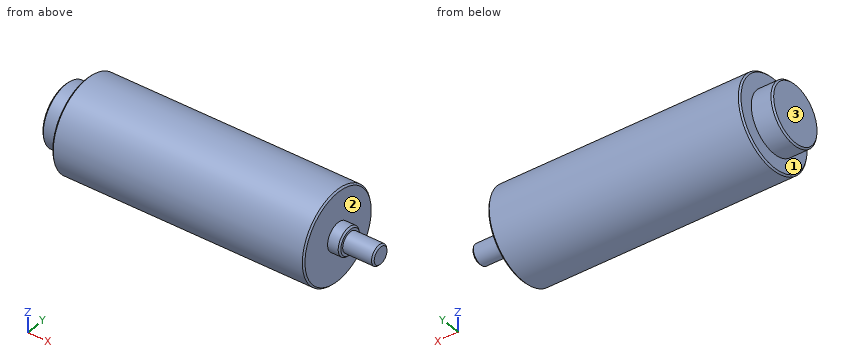
from build123d import *

# Parameters (mm, degrees)
CHAMFER1_SIZE = 0.5


with BuildPart() as part:
    # Sketch1 → Revolve1 (revolve)
    with BuildSketch(Plane.XY):
        Polygon((695.508784709, 30.649610335), (685.508784709, 30.649610335), (685.508784709, 31.949610335), (681.508784709, 31.949610335), (681.508784709, 42.349610335), (598.508784709, 42.349610335), (598.508784709, 37.349610335), (591.508784709, 37.349610335), (591.508784709, 27.349610335), (695.508784709, 27.349610335), align=None)
    revolve(axis=Axis((695.508784709, 27.349610335, 0), (-1, 0, 0)))

    # Chamfer1
    chamfer1_edges = [part.edges().sort_by_distance(p)[0] for p in [
        (695.508784709, 24.049610335, 0),
        (685.508784709, 22.749610335, 0),
        (681.508784709, 12.349610335, 0),
        (598.508784709, 12.349610335, 0),
        (591.508784709, 17.349610335, 0),
    ]]
    chamfer(chamfer1_edges, length=CHAMFER1_SIZE)


solid = part.part
Geometry check sheet. Reference: the model listing, model coordinates, mm. Face numbers are marked on the shaded views. A direction names the side the tool comes from. Give positions to 0.01 mm unless a question says otherwise; leave off trailing zeros. Loops run counter-clockwise (first coordinate to the right, second up) from the corner with the lowest first, then second, coordinate; pieces in that order, holes last.
(1) Thickness scan on L1, parallel to X at y = 25, z = 3; L2, parallel to Y at x = 661.5, z = -0.5; L3, parallel to X at y = 21.5, z = -12.5. Record the ranges inside material, lowest first.
From the geometry:
L1: x = 591.51 to 685.51
L2: y = 12.36 to 42.34
L3: x = 598.51 to 681.51
(2) Set-up check for the marked faces 1, 2 and 3: record each of +Z, -Z, +X, -X, +Y, -Y from which the full face is reachable in a straight line by a thin tool's end or side.
From the geometry:
face 1: -X
face 2: +X
face 3: +Z, -Z, -X, +Y, -Y
(3) Depth check by flat-ended pin: pin 1 Ø2 at (x, y) = (655, 29.5) entering from -Z; pin 2 Ø1 at (x, y) = (672.5, 36.5) entering from -Z; pin 3 Ø1.5 at (x, z) = (652, 11.5) entering from -Y. Enter the tip coordinate at first touch or a pass-through.
From the geometry:
pin 1: stops at z = -14.96
pin 2: stops at z = -12.25
pin 3: stops at y = 16.89
(4) Section check A-A on z = 0. Record the cut outline in (x, y), then the cut area to 3 significant figures.
From the geometry:
outline: (591.51, 17.85) - (592.01, 17.35) - (598.51, 17.35) - (598.51, 12.85) - (599.01, 12.35) - (681.01, 12.35) - (681.51, 12.85) - (681.51, 22.75) - (685.01, 22.75) - (685.51, 23.25) - (685.51, 24.05) - (695.01, 24.05) - (695.51, 24.55) - (695.51, 30.15) - (695.01, 30.65) - (685.51, 30.65) - (685.51, 31.45) - (685.01, 31.95) - (681.51, 31.95) - (681.51, 41.85) - (681.01, 42.35) - (599.01, 42.35) - (598.51, 41.85) - (598.51, 37.35) - (592.01, 37.35) - (591.51, 36.85) - close
area: 2,730 mm2
(5) Section check B-B on x = 663.5. Record the cut outline in (y, z).
From the geometry:
outline: circle Ø30 at (27.35, 0)
